Part model, mm, in its own coordinate system. Face numbers are marked on the shaded views. A direction names the side the tool comes from. Coordinates: 2 decimals unless noted, no trailing zeros. Order: outer loops, then holes, each group sorted by start corner. A loop starts at its lowest first (then second) coordinate and runs counter-clockwise, first axis right, second up. Notation, with made-up numbers: M -29,-39 L -9,-39 A27 ccw -9,-5 Z; hole C 86,13.5 d9. An arc over 180 degrees is marked long. Answer in a Markdown table with one row per item. Add a question column.
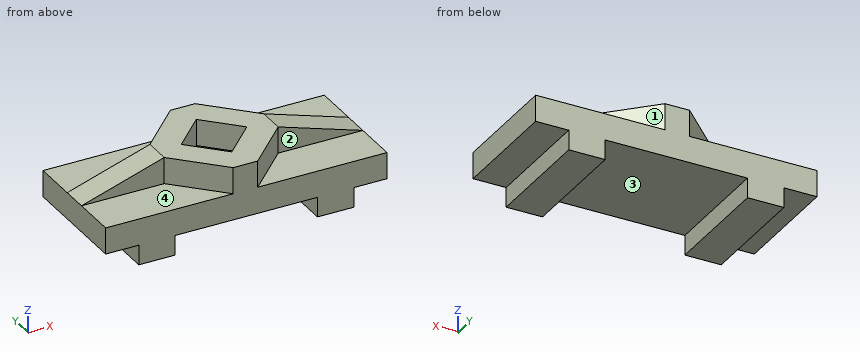
from build123d import *

# Parameters (mm, degrees)
BASE_PLATE_SKETCH_W      = 170
BASE_PLATE_SKETCH_H      = 70
BASE_PLATE_16MM_DEPTH    = 16
CENTER_BOSS_60X60_DEPTH  = 16
CENTER_POCKET_28_DEPTH   = 16
LEFT_WEDGE_BOSS_DEPTH    = 43
LEFT_WEDGE_CUT_DEPTH     = 27
RIGHT_WEDGE_BOSS_DEPTH   = 43
RIGHT_WEDGE_CUT_DEPTH    = 27
TOP_RAIL_SKETCH_W        = 22
TOP_RAIL_SKETCH_H        = 12
TOP_RAIL_WITH_TABS_DEPTH = 70


with BuildPart() as part:
    # Base Plate Sketch → Base Plate 16mm (new body)
    with BuildSketch(Plane.XY):
        with Locations((85, 35)):
            Rectangle(BASE_PLATE_SKETCH_W, BASE_PLATE_SKETCH_H)
    extrude(amount=BASE_PLATE_16MM_DEPTH)

    # Center Boss Sketch → Center Boss 60x60 (add)
    with BuildSketch(Plane.XY.offset(16)):
        Polygon((91.852813742, 70), (85, 70), (77, 70), (50, 43), (50, 35), (50, 27), (77, 0), (85, 0), (91.852813742, 0), (118.852813742, 27), (118.852813742, 35), (118.852813742, 43), align=None)
    extrude(amount=CENTER_BOSS_60X60_DEPTH)

    # Center Pocket Sketch → Center Pocket 28 (cut)
    with BuildSketch(Plane.XY.offset(32)):
        Polygon((84.426406871, 15.201010127), (104.225396744, 35), (84.426406871, 54.798989873), (64.627416998, 35), align=None)
    extrude(amount=-CENTER_POCKET_28_DEPTH, mode=Mode.SUBTRACT)

    # Left Wedge Sketch → Left Wedge Boss (add)
    with BuildSketch(Plane.XZ):
        Polygon((118.852813742, 32), (118.852813742, 16), (170, 16), align=None)
    extrude(amount=-LEFT_WEDGE_BOSS_DEPTH)

    # Left Wedge Cut Sketch → Left Wedge Cut (cut)
    with BuildSketch(Plane.XZ):
        Polygon((118.852813742, 32), (118.852813742, 16), (170, 16), align=None)
    extrude(amount=-LEFT_WEDGE_CUT_DEPTH, mode=Mode.SUBTRACT)

    # Right Wedge Sketch → Right Wedge Boss (add)
    with BuildSketch(Plane.XZ):
        Polygon((50, 32), (50, 16), (0, 16), align=None)
    extrude(amount=-RIGHT_WEDGE_BOSS_DEPTH)

    # Right Wedge Cut Sketch → Right Wedge Cut (cut)
    with BuildSketch(Plane.XZ):
        Polygon((50, 32), (50, 16), (0, 16), align=None)
    extrude(amount=-RIGHT_WEDGE_CUT_DEPTH, mode=Mode.SUBTRACT)

    # Top Rail Sketch → Top Rail with Tabs (add)
    with BuildSketch(Plane.XZ):
        with Locations((31, -6)):
            Rectangle(TOP_RAIL_SKETCH_W, TOP_RAIL_SKETCH_H)
        with Locations((139, -6)):
            Rectangle(TOP_RAIL_SKETCH_W, TOP_RAIL_SKETCH_H)
    extrude(amount=-TOP_RAIL_WITH_TABS_DEPTH)


solid = part.part
(1) Slice it at A-A (z = -6.5). List the corners of the cut face in (x, y).
(2) 3-axis set-ups, long thin cutter, end or side, ignore diameter. For the marked faces 1, 2, 3 and 4: which of +Z, -Z, +X, -X, +Y, -Y reach the whole face in a straight line?
(3) Drop flat-ended pins along their axis: P1, Ø5, axis at x = 153, z = 21.5, coming from the -Y side; P2, Ø13.5, axis at x = 21, y = 17.5, coming from the +Z side; P3, Ø9.5, axis at y = 37.5, z = -8.5, coming from the -X side; P4, Ø8, axis at x = 107.5, z = -4.5, coming from the +Y side. Give the stop position or say it passes through.
(4) Slice it at D-D (z = 19). List the corners of the cut face in (x, y) (3 decimals), and give its area (3 significant figures).
(5) Wall check: line 1 (X direction, y = 46, z = -3); line 2 (Z direction, x = 146.5, y = 65.5); line 3 (Y direction, x = 50, z = 27). Give the ranges that are in metal, low to high.
(6) Slice it at C-C (y = 66). List the corners of the cut face in (x, z).
(7) Slice it at B-B (x = 32.5). List the corners of the cut face in (y, z), and give its area (3 significant figures).
Computed:
| question | item | result |
|---|---|---|
| 1 | outline | M 20,0 L 42,0 L 42,70 L 20,70 Z; M 128,0 L 150,0 L 150,70 L 128,70 Z |
| 2 | face 1 | +Z, +X, +Y |
| 2 | face 2 | +Z, +X, -Y |
| 2 | face 3 | -Z, +Y, -Y |
| 2 | face 4 | +Z, -X, -Y |
| 3 | P1 | stops at y = 27 |
| 3 | P2 | stops at z = 16 |
| 3 | P3 | stops at x = 20 |
| 3 | P4 | passes through |
| 4 | outline | M 9.375,27 L 50,27 L 77,0 L 91.853,0 L 118.853,27 L 160.41,27 L 160.41,43 L 118.853,43 L 91.853,70 L 77,70 L 50,43 L 9.375,43 Z; hole M 64.627,35 L 84.426,15.201 L 104.225,35 L 84.426,54.799 Z |
| 4 | area | 3,890 mm^2 |
| 5 | line 1 | x = 20 to 42, 128 to 150 |
| 5 | line 2 | z = -12 to 16 |
| 5 | line 3 | y = 27 to 43 |
| 6 | outline | M 0,0 L 20,0 L 20,-12 L 42,-12 L 42,0 L 128,0 L 128,-12 L 150,-12 L 150,0 L 170,0 L 170,16 L 95.85,16 L 95.85,32 L 73,32 L 73,16 L 0,16 Z |
| 7 | outline | M 0,-12 L 70,-12 L 70,16 L 43,16 L 43,26.4 L 27,26.4 L 27,16 L 0,16 Z |
| 7 | area | 2,130 mm^2 |
